Build history of the part. All positions in model axes, mm. A direction names the side the tool comes from. Give positions to 0.01 mm unless a question says otherwise; leave off trailing zeros. Order: outer loops, then holes, each group sorted by start corner. A loop starts at its lowest first (then second) coordinate and runs counter-clockwise, first axis right, second up. Notation, with made-up numbers: (-20, -14) - (22, -14) arc R25 cw to (22, 19) - close; hole circle Ø7 at (48, 87). An arc over 180 degrees is marked (long way). Use a Markdown table: item, result. Add a question column.
(1) Wall check: line 1 (X direction, y = 6, z = 9.5); line 2 (X direction, y = -6.5, z = 2); line 3 (X direction, y = 2.75, z = 10). Give the ranges that are in metal, low to high.
(2) Mould opens along X. For faces 1 (the face through (55, 10.5, 9)), 2 (the face through (110, 0, 9)), 3 (the face through (-56.315, -5.838, 6.121)), 4 (the face through (-110, 0, 9)) say: +X half, -X half, draft (parallel to the pull), parting line (faces both ways), or undercut.
(3) Slice it at A-A (x = -100). Write the cut outline in (y, z), then the cut area to 3 significant figures.
(4) Flat gauge pins, fed straight in: pin 1 (5 mm diameter, centred on x = -24.5, z = 12, fed in from -Y); pin 2 (5 mm diameter, centred on x = 100, z = 9.5, fed in from +Y); pin 3 (3 mm diameter, centred on x = -97.5, z = 9, fed in from -Y); pin 4 (0.6 mm diameter, centred on x = -25.5, y = -9, fed in from +Z). Where does each tip first touch, or does it go through?
(5) Which spindle directions (+Z, -Z, +X, -X, +Y, -Y) get a long thin tool onto all of the face, cutting with end or side? Do faces 5 (the face through (2, -8.5, 10)), 6 (the face through (-102, -3.1, 12)), 7 (the face through (2.5, 8, 10)), 8 (the face through (97.253, 3.795, 9.379)). Say none if no direction does.
(6) Slice it at B-B (x = 68). Write the cut outline in (y, z).
from build123d import *

# Parameters (mm, degrees)
SKETCH_1_W                   = 220
SKETCH_1_H                   = 21
EXTRUDE_1_DEPTH              = 19
SKETCH_2_W                   = 220
SKETCH_2_H                   = 15
CUT_EXTRUDE_1_DEPTH          = 2
HOLE_WIZARD_M4_1_D           = 3.3
HOLE_WIZARD_M4_1_DEPTH       = 10.1
HOLE_WIZARD_M4_1_TIP         = 0.991420021
HOLE_WIZARD_M5_1_D           = 5.5
HOLE_WIZARD_M5_1_CBORE_D     = 10
HOLE_WIZARD_M5_1_CBORE_DEPTH = 5.4
SKETCH_7_W                   = 5
SKETCH_7_H                   = 5
CUT_EXTRUDE_2_DEPTH          = 113.12158579
HOLE_WIZARD_M3_1_D           = 2.5
HOLE_WIZARD_M3_1_DEPTH       = 7.5
HOLE_WIZARD_M3_1_TIP         = 0.751075774
SKETCH_12_W                  = 2
SKETCH_12_H                  = 2
CUT_EXTRUDE_3_DEPTH          = 222.06842832
CHAMFER_1_SIZE               = 0.5
HOLE_WIZARD_M3_2_D           = 2.5


with BuildPart() as part:
    # 草图1 → 凸台-拉伸1 (new body)
    with BuildSketch(Plane.XY):
        Rectangle(SKETCH_1_W, SKETCH_1_H)
    extrude(amount=EXTRUDE_1_DEPTH)

    # 草图2 → 切除-拉伸1 (cut)
    with BuildSketch(Plane.XZ.offset(10.5)):
        with Locations((0, 9.5)):
            Rectangle(SKETCH_2_W, SKETCH_2_H)
    extrude(amount=-CUT_EXTRUDE_1_DEPTH, mode=Mode.SUBTRACT)

    # M4 螺纹孔1
    with Locations(Plane(origin=(0, -8.5, 0), x_dir=(-1, 0, 0), z_dir=(0, -1, 0))):
        with Locations((-90, -9.5), (-30, -9.5), (30, -9.5), (90, -9.5)):
            Hole(HOLE_WIZARD_M4_1_D / 2, depth=HOLE_WIZARD_M4_1_DEPTH)
            with Locations((0, 0, -(HOLE_WIZARD_M4_1_DEPTH + HOLE_WIZARD_M4_1_TIP / 2))):  # 118° drill point
                Cone(0, HOLE_WIZARD_M4_1_D / 2, HOLE_WIZARD_M4_1_TIP, mode=Mode.SUBTRACT)

    # M5 六角凹头螺钉的柱形沉头孔1 (through all)
    with Locations(Plane(origin=(0, -8.5, 0), x_dir=(-1, 0, 0), z_dir=(0, -1, 0))):
        with Locations((-100, -9.5), (100, -9.5), (60, -9.5), (-60, -9.5)):
            CounterBoreHole(HOLE_WIZARD_M5_1_D / 2, HOLE_WIZARD_M5_1_CBORE_D / 2, HOLE_WIZARD_M5_1_CBORE_DEPTH)

    # 草图7 → 切除-拉伸2 (cut, through all)
    with BuildSketch(Plane.XY.offset(19)):
        with Locations((0, 8)):
            Rectangle(SKETCH_7_W, SKETCH_7_H)
    extrude(amount=-CUT_EXTRUDE_2_DEPTH, mode=Mode.SUBTRACT)

    # M3 螺纹孔1
    with Locations(Plane(origin=(0, 0, 0), x_dir=(-1, 0, 0), z_dir=(0, 0, -1))):
        with Locations((-55, -6.5), (0, -6.5)):
            Hole(HOLE_WIZARD_M3_1_D / 2, depth=HOLE_WIZARD_M3_1_DEPTH)
            with Locations((0, 0, -(HOLE_WIZARD_M3_1_DEPTH + HOLE_WIZARD_M3_1_TIP / 2))):  # 118° drill point
                Cone(0, HOLE_WIZARD_M3_1_D / 2, HOLE_WIZARD_M3_1_TIP, mode=Mode.SUBTRACT)

    # 草图12 → 切除-拉伸3 (cut, through all)
    with BuildSketch(Plane(origin=(110, 0, 0), x_dir=(0, 0, -1), z_dir=(1, 0, 0))):
        with Locations((-18, -9.5)):
            Rectangle(SKETCH_12_W, SKETCH_12_H)
    extrude(amount=-CUT_EXTRUDE_3_DEPTH, mode=Mode.SUBTRACT)

    # 倒角1
    chamfer_1_edges = [part.edges().sort_by_distance(p)[0] for p in [
        (-110, 1, 19),
        (110, 1, 19),
        (0, -8.5, 19),
        (110, -10.5, 1),
        (-110, -10.5, 1),
        (110, -8.5, 10.5),
        (110, -9.5, 2),
        (-110, -8.5, 10.5),
        (-110, -9.5, 2),
        (0, -10.5, 0),
        (-110, 0, 0),
        (56.25, 10.5, 0),
        (110, 0, 0),
        (56.25, 10.5, 19),
        (-110, 10.5, 9.5),
        (110, 10.5, 9.5),
        (-56.25, 10.5, 0),
        (-56.25, 10.5, 19),
    ]]
    chamfer(chamfer_1_edges, length=CHAMFER_1_SIZE)

    # M3 螺纹孔2 (through all)
    with Locations(Plane(origin=(0, 0, 0), x_dir=(-1, 0, 0), z_dir=(0, 0, -1))):
        with Locations((105, 0.5), (-105, 0.5)):
            Hole(HOLE_WIZARD_M3_2_D / 2)


solid = part.part
Solution:
| question | item | result |
|---|---|---|
| 1 | line 1 | -110 to -102.75, -97.25 to -62.75, -57.25 to -2.5, 2.5 to 57.25, 62.75 to 97.25, 102.75 to 110 |
| 1 | line 2 | -110 to -1.25, 1.25 to 53.75, 56.25 to 110 |
| 1 | line 3 | -110 to -102.7, -97.3 to -62.7, -57.3 to 57.3, 62.7 to 97.3, 102.7 to 110 |
| 2 | face 1 | draft |
| 2 | face 2 | +X half |
| 2 | face 3 | undercut |
| 2 | face 4 | -X half |
| 3 | outline | (-10.5, 0.5) - (-10, 0) - (10, 0) - (10.5, 0.5) - (10.5, 6.75) - (-3.1, 6.75) - (-3.1, 4.5) - (-8.5, 4.5) - (-8.5, 2) - (-10.5, 2) - close; (-8.5, 14.5) - (-3.1, 14.5) - (-3.1, 12.25) - (10.5, 12.25) - (10.5, 18.5) - (10, 19) - (-8, 19) - (-8.5, 18.5) - close |
| 3 | area | 236 mm2 |
| 4 | pin 1 | y = -8.5 |
| 4 | pin 2 | through |
| 4 | pin 3 | y = -3.1 |
| 4 | pin 4 | z = 2 |
| 5 | face 5 | +Z, +X, -X, -Y |
| 5 | face 6 | -Y |
| 5 | face 7 | +Z, -Z, +Y |
| 5 | face 8 | +Y, -Y |
| 6 | outline | (-10.5, 0.5) - (-10, 0) - (10, 0) - (10.5, 0.5) - (10.5, 18.5) - (10, 19) - (-8, 19) - (-8.5, 18.5) - (-8.5, 2) - (-10.5, 2) - close |
